Can you work these out from the drawing? Everything is in mm from the part's minimum corner. Coordinates: 2 decimals unless noted, no trailing zeros. Write each loop counter-clockwise with the first axis right and the second up, starting at its lowest first coordinate (ties: lowest second). Pieces come first, ordered by that corner, then holes. Notation, with made-up numbers: M 86,7.25 L 140,7.25 A15 cw 140,13.25 Z; hole C 54,-5 d11. An arc over 180 degrees is marked long. Answer as a JSON object with one key per item and string values. Group by question number.
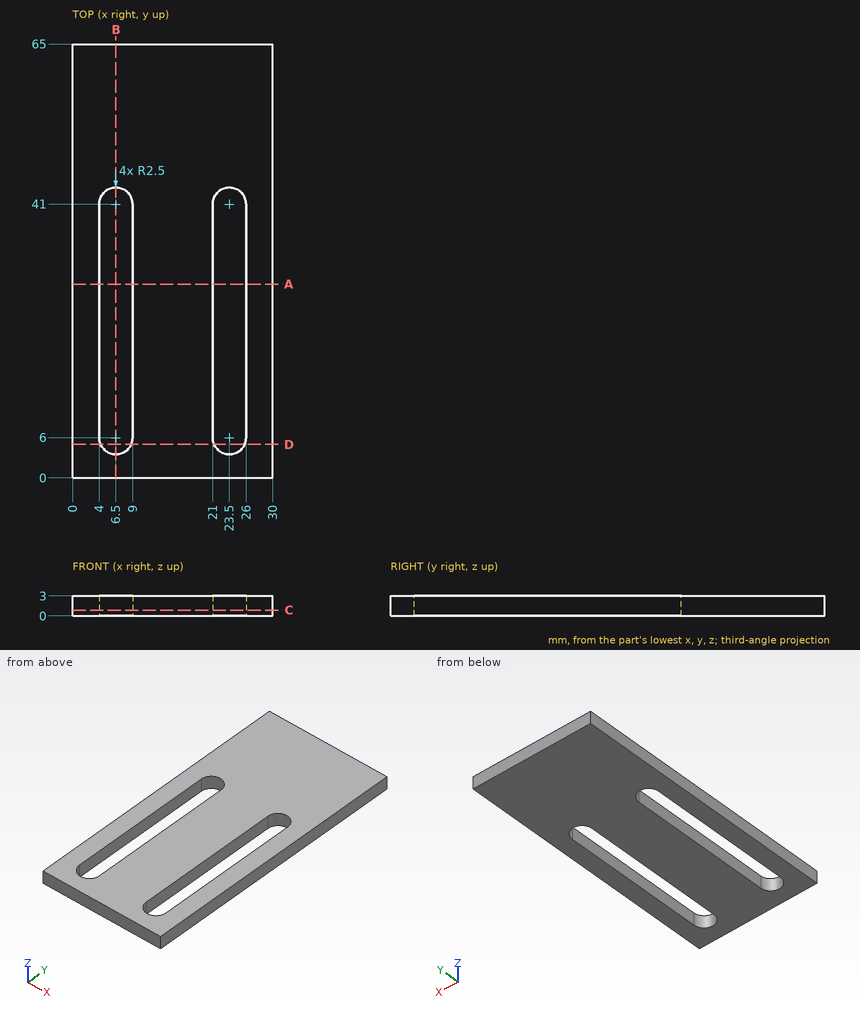
Q1. If we section it at A-A on y = 29: List the corners of the cut face in (x, z) for me.
Q2. If we section it at C-C on z = 0.85: List the corners of the cut face in (x, y) for me.
Q3. If we section it at B-B on x = 6.5: List the corners of the cut face in (y, z) for me, and give its area (3 significant figures).
Q4. Please list where these lines run through material, in increasing order: L1, parallel to X at y = 27, z = 2.05; L2, parallel to Y at x = 6.5, z = 1.6; L3, parallel to X at y = 43, z = 1.65.
Q5. If we section it at D-D on y = 5: List the corners of the cut face in (x, z) for me, and give its area (3 significant figures).
Reply:
{
 "1": {"outline": "M 0,0 L 4,0 L 4,3 L 0,3 Z; M 9,0 L 21,0 L 21,3 L 9,3 Z; M 26,0 L 30,0 L 30,3 L 26,3 Z"},
 "2": {"outline": "M 0,0 L 30,0 L 30,65 L 0,65 Z; hole M 4,6 A2.5 ccw 9,6 L 9,41 A2.5 ccw 4,41 Z; hole M 21,6 A2.5 ccw 26,6 L 26,41 A2.5 ccw 21,41 Z"},
 "3": {"outline": "M 0,0 L 3.5,0 L 3.5,3 L 0,3 Z; M 43.5,0 L 65,0 L 65,3 L 43.5,3 Z", "area": "75.0 mm^2"},
 "4": {"L1": "0 to 4, 9 to 21, 26 to 30", "L2": "0 to 3.5, 43.5 to 65", "L3": "0 to 5, 8 to 22, 25 to 30"},
 "5": {"outline": "M 0,0 L 4.21,0 L 4.21,3 L 0,3 Z; M 8.79,0 L 21.21,0 L 21.21,3 L 8.79,3 Z; M 25.79,0 L 30,0 L 30,3 L 25.79,3 Z", "area": "62.5 mm^2"}
}
